Work out the finished part from the listing and answer in its coordinate system (mm). Face numbers are marked on the shaded views. A direction names the side the tool comes from. Coordinates: 2 decimals unless noted, no trailing zeros. Order: outer loops, then holes, each group sorted by start corner. A loop starts at its lowest first (then second) coordinate and runs counter-clockwise, first axis right, second up. Notation, with made-up numbers: M -12,33 L 27,33 A14 cw 27,46 Z; hole C 29.25,-21 d4. An arc over 180 degrees is marked long. Use a Markdown table: item, result.
from build123d import *

# Parameters (mm, degrees)
BOSS_EXTRUDE1_DEPTH = 8
CUT_EXTRUDE1_DEPTH  = 10


with BuildPart() as part:
    # Sketch1 → Boss-Extrude1 (new body)
    with BuildSketch(Plane.XY):
        with BuildLine():
            Line((10, 0), (70, 0))
            ThreePointArc((70, 0), (77.071067812, 2.928932188), (80, 10))
            Line((80, 10), (80, 130))
            ThreePointArc((80, 130), (77.071067812, 137.071067812), (70, 140))
            Line((70, 140), (10, 140))
            ThreePointArc((10, 140), (2.928932188, 137.071067812), (0, 130))
            Line((0, 130), (0, 10))
            ThreePointArc((0, 10), (2.928932188, 2.928932188), (10, 0))
        make_face()
    extrude(amount=BOSS_EXTRUDE1_DEPTH)

    # Sketch2 → Cut-Extrude1 (cut)
    with BuildSketch(Plane.XY.offset(8)):
        with BuildLine():
            Line((34.5, 12), (34.5, 42))
            ThreePointArc((34.5, 42), (40, 47.5), (45.5, 42))
            Line((45.5, 42), (45.5, 12))
            ThreePointArc((45.5, 12), (40, 6.5), (34.5, 12))
        make_face()
    extrude(amount=-CUT_EXTRUDE1_DEPTH, mode=Mode.SUBTRACT)


solid = part.part
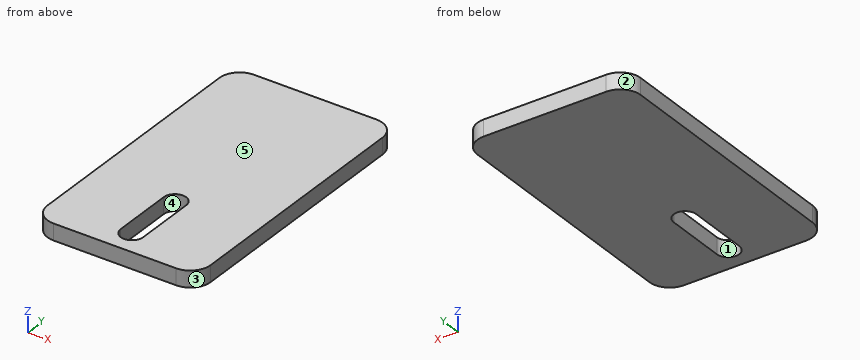
(1) A cutting plane is placed at A-A (x = 40). Determine the outline of the cut face in (y, z).
Conclusion:
| item | result |
|---|---|
| outline | M 0,0 L 6.5,0 L 6.5,8 L 0,8 Z; M 47.5,0 L 140,0 L 140,8 L 47.5,8 Z |
(2) Which of the six approach directions +Z, -Z, +X, -X, +Y, -Y give full straight-line access (tool end or side, diameter ignored) to the marked faces 1 and 2?
Conclusion:
| item | result |
|---|---|
| face 1 | +Z, -Z |
| face 2 | +Z, -Z, -X, +Y |
(3) Straight lines are drawn through the part: L1, parallel to X at y = 23.5, z = 6.75; L2, parallel to Y at x = 36, z = 4.25; L3, parallel to Y at x = 44.5, z = 3. For each, find the intervals that lie inside material, in ascending order.
Conclusion:
| item | result |
|---|---|
| L1 | 0 to 34.5, 45.5 to 80 |
| L2 | 0 to 8.23, 45.77 to 140 |
| L3 | 0 to 8.84, 45.16 to 140 |
(4) Determine the mould class of the marked faces 3, 4 and 5 for opening direction X: pulls with the +X half, pulls with the -X half, needs draft (parallel to the pull), parting line crosses it, or undercut.
Conclusion:
| item | result |
|---|---|
| face 3 | pulls with the +X half |
| face 4 | undercut |
| face 5 | needs draft |
(5) A cutting plane is placed at B-B (z = 1.75). Determine the outline of the cut face in (x, y), then the cut area to 3 significant figures.
Conclusion:
| item | result |
|---|---|
| outline | M 0,10 A10 ccw 10,0 L 70,0 A10 ccw 80,10 L 80,130 A10 ccw 70,140 L 10,140 A10 ccw 0,130 Z; hole M 34.5,12 A5.5 ccw 45.5,12 L 45.5,42 A5.5 ccw 34.5,42 Z |
| area | 10,700 mm2 |
